For this review, use the dimensioned drawing (mm, ordinates from the lowest corner) and the shaded views. Coordinates: 2 decimals unless noted, no trailing zeros. Loops run counter-clockwise (first coordinate to the right, second up) from the corner with the lowest first, then second, coordinate; pieces in that order, holes last. Notation, with made-up numbers: (-34, 51.5) - (18, 51.5) arc R18 cw to (18, 73.5) - close; hole circle Ø4 at (78, 17). An arc over 180 degrees is marked (long way). Answer in a Markdown table with one row per item. Add a question column.
(1) We need section D-D, the plane z = 18.75. Write out the cut boundary in (x, y) (3 decimals).
(2) We need section A-A, the plane y = 32.5. Write out the cut boundary in (x, z) (3 decimals), plus the area to 4 significant figures.
(3) To check wall thickness, follow L1, parallel to Z at x = 41, y = 3.5; L2, parallel to Y at x = 22.5, z = 12.5; L3, parallel to Y at x = 32.5, z = 7.75 (3 decimals). State the ranges of each line that lie inside material, in increasing order. Write a range as [from, to].
(4) We need section C-C, the plane z = 2. Write out the cut boundary in (x, y) (3 decimals), plus the area to 3 significant figures.
(5) The part is to be moulded in two halves that separate along Y. For the marked faces 1, 2 and 3, say which applies: released by +Y, released by -Y, zero draft, split by the parting line, or undercut.
(6) Clearance check with flat-ended pins moving along their axes: pin 1 (1 mm diameter, centred on y = 24.5, z = 16, fed in from -X); pin 2 (4 mm diameter, centred on y = 40, z = 8, fed in from -X); pin 3 (1.5 mm diameter, centred on y = 15.5, z = 11.5, fed in from -X). State where each tip first meets the part, or that it passes through.
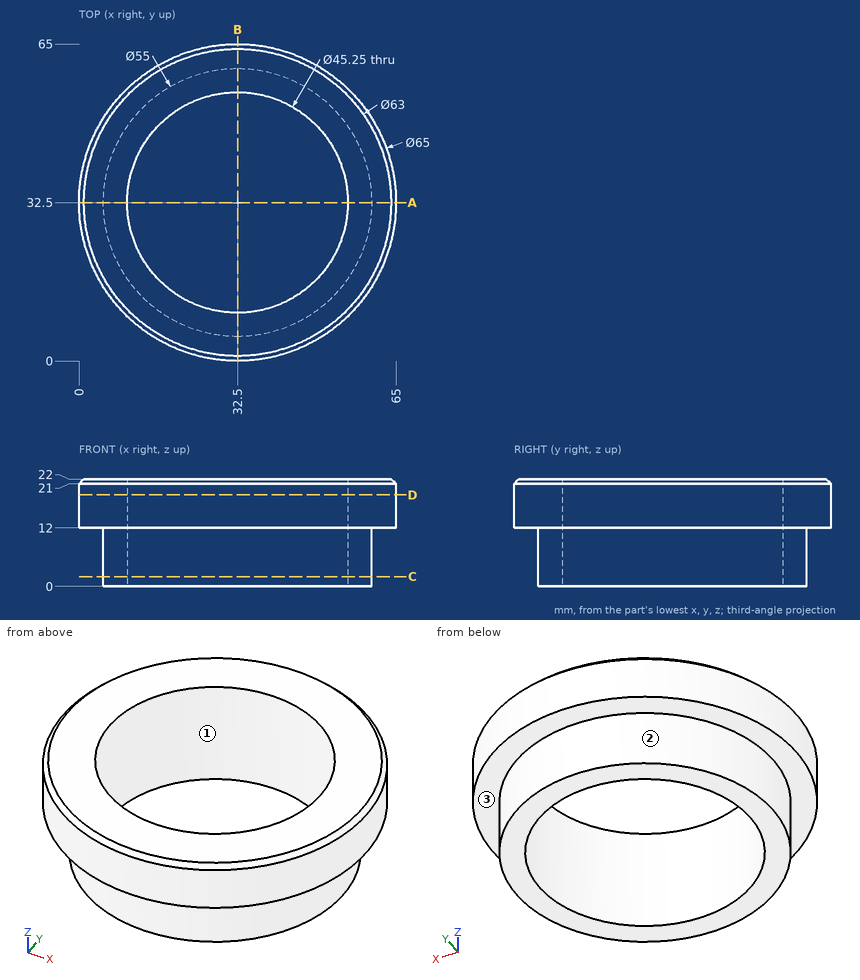
Responses:
| question | item | result |
|---|---|---|
| 1 | outline | circle Ø65 at (32.5, 32.5); hole circle Ø45.25 at (32.5, 32.5) |
| 2 | outline | (0, 12) - (5, 12) - (5, 0) - (9.875, 0) - (9.875, 22) - (1, 22) - (0, 21) - close; (55.125, 0) - (60, 0) - (60, 12) - (65, 12) - (65, 21) - (64, 22) - (55.125, 22) - close |
| 2 | area | 313.5 mm2 |
| 3 | L1 | z = [12, 22] |
| 3 | L2 | y = [1.58, 12.2], [52.8, 63.42] |
| 3 | L3 | y = [5, 9.875], [55.125, 60] |
| 4 | outline | circle Ø55 at (32.5, 32.5); hole circle Ø45.25 at (32.5, 32.5) |
| 4 | area | 768 mm2 |
| 5 | face 1 | undercut |
| 5 | face 2 | split by the parting line |
| 5 | face 3 | zero draft |
| 6 | pin 1 | stops at x = 0.88 |
| 6 | pin 2 | stops at x = 5.56 |
| 6 | pin 3 | stops at x = 4.47 |
